The drawing under review shows one solid part. Ordinate dimensions are in mm from its lowest x, y, z. A direction names the side the tool comes from. Give positions to 0.01 mm unless a question says otherwise; leave off trailing zeros. Loops run counter-clockwise (first coordinate to the right, second up) from the corner with the lowest first, then second, coordinate; pieces in that order, holes last.
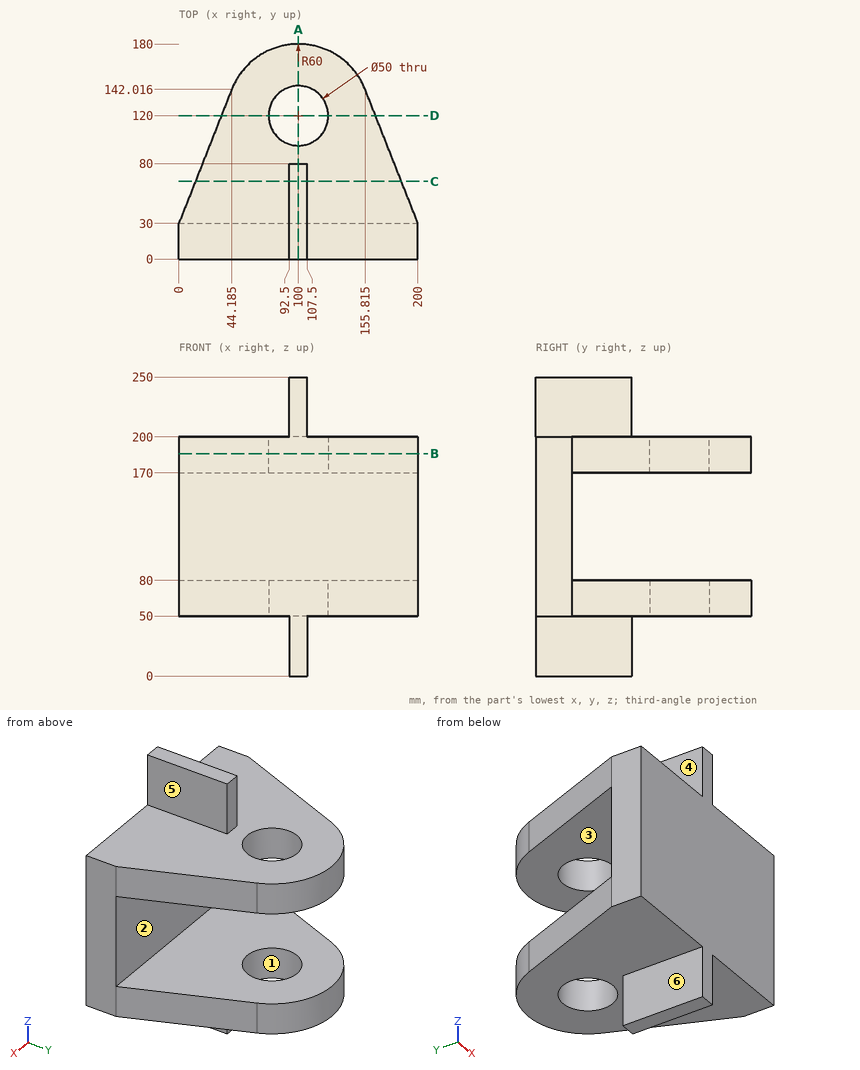
Item 1: The part is to be moulded in two halves that separate along Z. For the marked faces 1 and 2, say which applies: released by +Z, released by -Z, zero draft, split by the parting line, or undercut.
Answer:
face 1: zero draft
face 2: undercut
Item 2: Take a section at C-C on y = 65. Give the boundary of the cut face in (x, z), and give its area (3 significant figures).
Answer:
outline: (13.81, 50) - (92.5, 50) - (92.5, 0) - (107.5, 0) - (107.5, 50) - (186.19, 50) - (186.19, 80) - (13.81, 80) - close; (13.81, 170) - (186.19, 170) - (186.19, 200) - (107.5, 200) - (107.5, 250) - (92.5, 250) - (92.5, 200) - (13.81, 200) - close
area: 11,800 mm2
Item 3: Clearance check with flat-ended pins moving along their axes: pin 1 Ø12 at (x, y) = (153.5, 92) entering from +Z; pin 2 Ø10 at (x, z) = (158.5, 103) entering from +Y; pin 3 Ø4.5 at (x, z) = (99.5, 233) entering from +Y. State where each tip first meets the part, or that it passes through.
Answer:
pin 1: stops at z = 200
pin 2: stops at y = 30
pin 3: stops at y = 80
Item 4: Tool access review of the marked faces 3, 4, 5 and 6: name each direction out of +Z, -Z, +X, -X, +Y, -Y from which nothing blocks a thin tool from reaching the whole face with its end or side.
Answer:
face 3: +X, -X, +Y
face 4: +Z, -X, +Y, -Y
face 5: +Z, +X, +Y, -Y
face 6: -Z, -X, +Y, -Y
Item 5: For L1, parallel to Z at x = 137, y = 65; L2, parallel to Y at x = 14, z = 101; L3, parallel to X at y = 118, z = 79, list the stretches that pass through material, from the lowest coordinate up.
Answer:
L1: z = 50 to 80, 170 to 200
L2: y = 0 to 30
L3: x = 34.71 to 75.08, 124.92 to 165.29
Item 6: Take a section at A-A on x = 100. Give the boundary of the cut face in (y, z), and give its area (3 significant figures).
Answer:
outline: (0, 0) - (80, 0) - (80, 50) - (95, 50) - (95, 80) - (30, 80) - (30, 170) - (95, 170) - (95, 200) - (80, 200) - (80, 250) - (0, 250) - close; (145, 50) - (180, 50) - (180, 80) - (145, 80) - close; (145, 170) - (180, 170) - (180, 200) - (145, 200) - close
area: 18,500 mm2
Item 7: Take a section at D-D on y = 120. Give the boundary of the cut face in (x, z).
Answer:
outline: (35.5, 50) - (75, 50) - (75, 80) - (35.5, 80) - close; (35.5, 170) - (75, 170) - (75, 200) - (35.5, 200) - close; (125, 50) - (164.5, 50) - (164.5, 80) - (125, 80) - close; (125, 170) - (164.5, 170) - (164.5, 200) - (125, 200) - close
Item 8: Take a section at B-B on z = 186. Give the boundary of the cut face in (x, y) (1 decimal), and give its area (3 significant figures).
Answer:
outline: (0, 0) - (200, 0) - (200, 30) - (155.8, 142) arc R60 ccw to (44.2, 142) - (0, 30) - close; hole circle Ø50 at (100, 120)
area: 24,600 mm2
